Work out the finished part from the listing and answer in its coordinate system (mm). Coordinates: 2 decimals unless noted, no trailing zeros. Order: outer loops, then holes, each group sorted by start corner. A loop starts at its lowest first (then second) coordinate and runs counter-clockwise, first axis right, second up. Notation, with made-up numbers: (-10, 14) - (36, 14) arc R21 ccw to (36, 49) - close; hole circle Ø7 at (82.5, 61.5). An arc over 180 degrees is marked (long way). Answer as a JSON object with one key per item and string values. Group by question number.
1) Section A-A (z = 0) is taken. Give the vertices of the cut face in (x, y), plus the area to 3 significant figures.
2) Section B-B (x = 0) is taken. Give the vertices of the cut face in (y, z).
3) Section C-C (y = -944) is taken. Give the vertices of the cut face in (x, z), plus the area to 3 significant figures.
4) Find the intervals of material crossed by line 1 along Z through (x, y) = (-2.25, -663); line 2 along Z through (x, y) = (10, -76); line 3 along Y through (x, z) = (7.25, 5), in increasing order.
5) Each of these flat-tipped pins is pushed along its axis until it touches: P1, Ø6, axis at x = -5, y = -598, coming from the +Z side; P2, Ø10, axis at x = -6, y = -441, coming from the +Z side; P3, Ø1.5, axis at y = -577.5, z = 9, coming from the +X side; P4, Ø10, axis at x = -8, z = -8, coming from the -Y side. Where does it stop, or does it pass through?
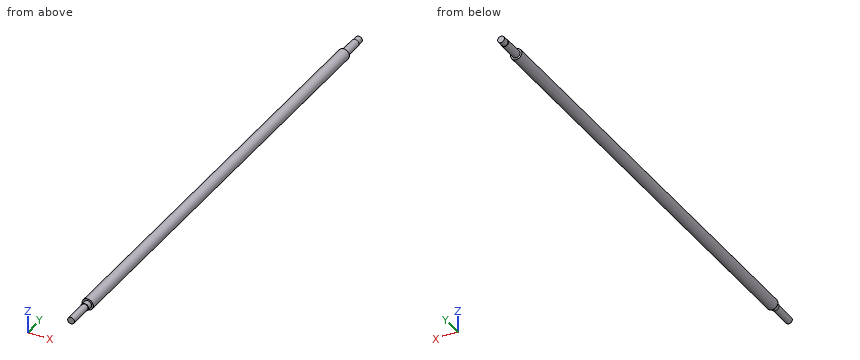
from build123d import *


with BuildPart() as part:
    # Sketch2 → Revolve1 (revolve)
    with BuildSketch(Plane.XY, mode=Mode.PRIVATE) as revolve1_sk:
        Polygon((0, 0), (7.5, 0), (7.5, -15), (8.5, -15), (8.5, -61), (12.5, -61), (12.5, -1090), (8.5, -1090), (8.5, -1102), (7.5, -1102), (7.5, -1157), (0, -1157), align=None)
    revolve(revolve1_sk.sketch.rotate(Axis((0, 0, 0), (0, 1, 0)), 90), axis=Axis((0, 0, 0), (0, 1, 0)))


solid = part.part
Report:
{
 "1": {"outline": "(-12.5, -1090) - (-8.5, -1090) - (-8.5, -1102) - (-7.5, -1102) - (-7.5, -1157) - (7.5, -1157) - (7.5, -1102) - (8.5, -1102) - (8.5, -1090) - (12.5, -1090) - (12.5, -61) - (8.5, -61) - (8.5, -15) - (7.5, -15) - (7.5, 0) - (-7.5, 0) - (-7.5, -15) - (-8.5, -15) - (-8.5, -61) - (-12.5, -61) - close", "area": "27,800 mm²"},
 "2": {"outline": "(-1157, -7.5) - (-1102, -7.5) - (-1102, -8.5) - (-1090, -8.5) - (-1090, -12.5) - (-61, -12.5) - (-61, -8.5) - (-15, -8.5) - (-15, -7.5) - (0, -7.5) - (0, 7.5) - (-15, 7.5) - (-15, 8.5) - (-61, 8.5) - (-61, 12.5) - (-1090, 12.5) - (-1090, 8.5) - (-1102, 8.5) - (-1102, 7.5) - (-1157, 7.5) - close"},
 "3": {"outline": "circle Ø25 at (0, 0)", "area": "491 mm²"},
 "4": {"line 1": "z = -12.3 to 12.3", "line 2": "z = -7.5 to 7.5", "line 3": "y = -1090 to -61"},
 "5": {"P1": "stops at z = 12.34", "P2": "stops at z = 12.46", "P3": "stops at x = 9.39", "P4": "stops at y = -1157"}
}
